The listing builds one solid part. Answer for the finished solid, in the listing's coordinates (mm). Face numbers are marked on the shaded views. A direction names the side the tool comes from. Coordinates: 2 decimals unless noted, no trailing zeros. Write each loop counter-clockwise with the first axis right and the second up, starting at its lowest first coordinate (ties: lowest second). Pieces come first, ordered by that corner, then holes.
from build123d import *

# Parameters (mm, degrees)
SKETCH_1_W                   = 18
SKETCH_1_H                   = 65.5
EXTRUDE_1_DEPTH              = 6
SKETCH_2_W                   = 28
SKETCH_2_H                   = 35
EXTRUDE_2_DEPTH              = 12
CUT_EXTRUDE_1_DEPTH          = 40.71854101
SKETCH_4_W                   = 18
SKETCH_4_H                   = 12
EXTRUDE_3_DEPTH              = 70
CHAMFER_1_SIZE               = 10
HOLE_WIZARD_M6_1_D           = 6.6
HOLE_WIZARD_M6_1_CBORE_D     = 11
HOLE_WIZARD_M6_1_CBORE_DEPTH = 6.4
F_6_0MM_1_D                  = 6
CHAMFER_2_SIZE               = 1


with BuildPart() as part:
    # 草图1 → 凸台-拉伸1 (new, symmetric)
    with BuildSketch(Plane.XY):
        Rectangle(SKETCH_1_W, SKETCH_1_H)
    extrude(amount=EXTRUDE_1_DEPTH, both=True)

    # 草图2 → 凸台-拉伸2 (add)
    with BuildSketch(Plane.XY.offset(6)):
        with Locations((-5, -15.25)):
            Rectangle(SKETCH_2_W, SKETCH_2_H)
    extrude(amount=-EXTRUDE_2_DEPTH)

    # 草图3 → 切除-拉伸1 (cut, through all)
    with BuildSketch(Plane.XY.offset(6)):
        with BuildLine():
            Line((-3, -9), (21, -9))
            ThreePointArc((21, -9), (28.75, -16.75), (21, -24.5))
            Line((21, -24.5), (-3, -24.5))
            ThreePointArc((-3, -24.5), (-10.75, -16.75), (-3, -9))
        make_face()
    extrude(amount=-CUT_EXTRUDE_1_DEPTH, mode=Mode.SUBTRACT)

    # 草图4 → 凸台-拉伸3 (add)
    with BuildSketch(Plane(origin=(0, 0, -6), x_dir=(-1, 0, 0), z_dir=(0, 0, -1))):
        with Locations((0, 26.75)):
            Rectangle(SKETCH_4_W, SKETCH_4_H)
    extrude(amount=EXTRUDE_3_DEPTH)

    # 倒角1
    chamfer_1_edges = [part.edges().sort_by_distance(p)[0] for p in [
        (0, 20.75, -6),
    ]]
    chamfer(chamfer_1_edges, length=CHAMFER_1_SIZE)

    # M6 六角凹头螺钉的柱形沉头孔1 (through all)
    with Locations(Plane(origin=(0, 20.75, 0), x_dir=(-1, 0, 0), z_dir=(0, -1, 0))):
        with Locations((0, 23), (0, 70)):
            CounterBoreHole(HOLE_WIZARD_M6_1_D / 2, HOLE_WIZARD_M6_1_CBORE_D / 2, HOLE_WIZARD_M6_1_CBORE_DEPTH)

    # Ø6.0mm 暗销孔1 (through all)
    with Locations(Plane(origin=(0, 20.75, 0), x_dir=(-1, 0, 0), z_dir=(0, -1, 0))):
        with Locations((0, 36.5), (0, 56.5)):
            Hole(F_6_0MM_1_D / 2)

    # 倒角2
    chamfer_2_edges = [part.edges().sort_by_distance(p)[0] for p in [
        (-19, 2.25, 0),
        (-19, -32.75, 0),
        (9, -9, 0),
        (9, -24.5, 0),
        (-9, 26.75, -76),
        (9, 26.75, -76),
        (9, -32.75, 0),
    ]]
    chamfer(chamfer_2_edges, length=CHAMFER_2_SIZE)


solid = part.part
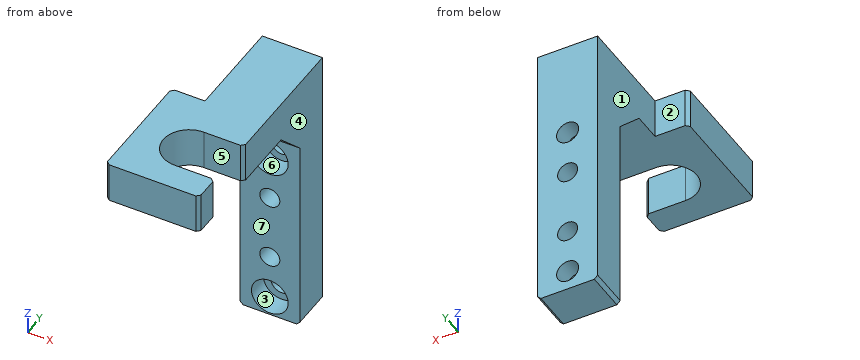
1. Section A-A on z = -56.5 is taken. Give the vertices of the cut face in (x, y).
Results found:
outline: (-9, 20.75) - (-3, 20.75) - (-3, 32.75) - (-9, 32.75) - close; (3, 20.75) - (9, 20.75) - (9, 32.75) - (3, 32.75) - close
2. A tool of negligible diameter and unlimited length cuts with its end or side. For the marked faces 4, 5, 6 and 7, from which of +Z, -Z, +X, -X, +Y, -Y can it reach the whole face along a straight path? Write none if from no direction.
Results found:
face 4: +Z, -Z, +X, +Y, -Y
face 5: +Z, -Z, +X
face 6: -Y
face 7: -Z, +X, -X, -Y
3. Section B-B on x = 4.25 is taken. Give the vertices of the cut face in (y, z).
Results found:
outline: (-32.75, -6) - (-24.5, -6) - (-24.5, 6) - (-32.75, 6) - close; (-9, -6) - (10.75, -6) - (20.75, -16) - (20.75, -19.51) - (27.15, -19.51) - (27.15, -26.49) - (20.75, -26.49) - (20.75, -66.51) - (27.15, -66.51) - (27.15, -73.49) - (20.75, -73.49) - (20.75, -76) - (32.75, -76) - (32.75, 6) - (-9, 6) - close
4. Find the intervals of material crossed by L1, parallel to Z at x = 0, y = 23.5; L2, parallel to Y at x = 3.25, z = -0.5; L3, parallel to Z at x = 0, y = 30.25, in increasing order.
Results found:
L1: z = -76 to -75.5, -64.5 to -59.5, -53.5 to -39.5, -33.5 to -28.5, -17.5 to 6
L2: y = -32.75 to -24.5, -9 to 32.75
L3: z = -76 to -73.3, -66.7 to -59.5, -53.5 to -39.5, -33.5 to -26.3, -19.7 to 6
5. Section C-C on y = -16.75 is taken. Give the vertices of the cut face in (x, z).
Results found:
outline: (-19, -6) - (-10.75, -6) - (-10.75, 6) - (-19, 6) - close
6. Flat-ended cylindrical pins translate along their axes: P1, Ø5.5, axis at x = 0, z = -23, coming from the -Y side; P2, Ø7, axis at x = 0, z = -56.5, coming from the -Y side; P3, Ø6, axis at x = 0, y = 12.5, coming from the -Z side; P4, Ø10.5, axis at x = 0, z = -70, coming from the -Y side. Find the tip coordinate at first contact, or state that the pin passes through.
Results found:
P1: passes through
P2: stops at y = 20.75
P3: stops at z = -10.75
P4: stops at y = 27.15
7. Section D-D on z = -70 is taken. Give the vertices of the cut face in (x, y), then the cut area to 3 significant figures.
Results found:
outline: (-9, 20.75) - (-5.5, 20.75) - (-5.5, 27.15) - (-3.3, 27.15) - (-3.3, 32.75) - (-9, 32.75) - close; (3.3, 27.15) - (5.5, 27.15) - (5.5, 20.75) - (9, 20.75) - (9, 32.75) - (3.3, 32.75) - close
area: 109 mm2
8. For a pull along X with two mould halves and no side action, classify the marked faces 1, 2 and 3 as pulls with the +X half, pulls with the -X half, needs draft (parallel to the pull), parting line crosses it, or undercut.
Results found:
face 1: pulls with the -X half
face 2: needs draft
face 3: undercut
